Source: CAD feature listing. Evaluate the final solid. Frame: model axes, mm. Face numbers are marked on the shaded views. Give positions to 0.01 mm unless a question says otherwise; leave off trailing zeros. Order: outer loops, then holes, each group sorted by start corner. A loop starts at its lowest first (then second) coordinate and runs counter-clockwise, first axis right, second up.
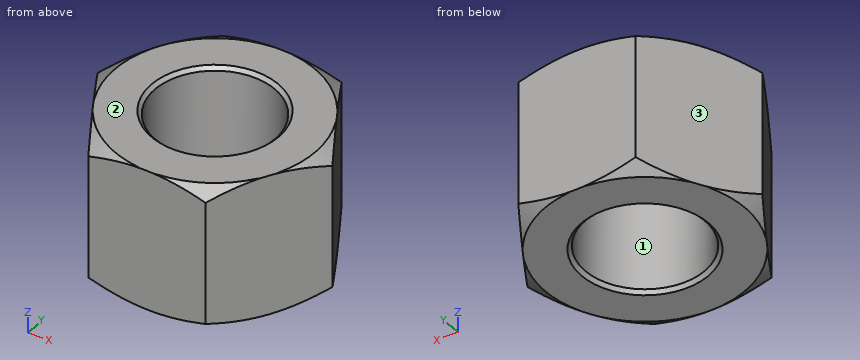
```python
from build123d import *

# Parameters (mm, degrees)
SKETCH1_R          = 5.9175
BOSS_EXTRUDE_DEPTH = 13.9
SKETCH2_OUTSIDE_W  = 105.954
SKETCH2_OUTSIDE_H  = 102.9
SKETCH2_OUTSIDE_R  = 9.872689603
CUT_EXTRUDE1_DEPTH = 21.509509989
CUT_EXTRUDE1_DRAFT = -60
SKETCH3_OUTSIDE_W  = 105.954
SKETCH3_OUTSIDE_H  = 102.9
SKETCH3_OUTSIDE_R  = 9.872689603
CUT_EXTRUDE2_DEPTH = 21.509509989
CUT_EXTRUDE2_DRAFT = -60
CHAMFER1_SIZE      = 0.3475


with BuildPart() as part:
    # Sketch1 → Boss-Extrude (new body)
    with BuildSketch(Plane.XY):
        Polygon((5.7, 9.872689603), (-5.7, 9.872689603), (-11.4, 0), (-5.7, -9.872689603), (5.7, -9.872689603), (11.4, 0), align=None)
        Circle(SKETCH1_R, mode=Mode.SUBTRACT)
    extrude(amount=BOSS_EXTRUDE_DEPTH)


with BuildPart() as cut_extrude1_tool:
    # Sketch2 outside → Cut-Extrude1 (with draft: the straight prism first)
    with BuildSketch(Plane(origin=(0, 0, 0), x_dir=(-1, 0, 0), z_dir=(0, 0, -1))):
        Rectangle(SKETCH2_OUTSIDE_W, SKETCH2_OUTSIDE_H)
        Circle(SKETCH2_OUTSIDE_R, mode=Mode.SUBTRACT)
    extrude(amount=-CUT_EXTRUDE1_DEPTH)
    # Cut-Extrude1: the draft: its side faces are tilted about the plane it starts from
    cut_extrude1_sides = [cut_extrude1_tool.faces().sort_by_distance(p)[0] for p in [
        (0, -51.45, 10.754754995),
        (-52.977, 0, 10.754754995),
        (0, 51.45, 10.754754995),
        (52.977, 0, 10.754754995),
        (9.872689603, 0, 10.754754995),
    ]]
    draft(cut_extrude1_sides, Plane(origin=(0, 0, 0), x_dir=(-1, 0, 0), z_dir=(0, 0, -1)), CUT_EXTRUDE1_DRAFT)


with BuildPart() as part_1:
    add(part.part)

    # Cut-Extrude1: cut by cut_extrude1_tool
    add(cut_extrude1_tool.part, mode=Mode.SUBTRACT)


with BuildPart() as cut_extrude2_tool:
    # Sketch3 outside → Cut-Extrude2 (with draft: the straight prism first)
    with BuildSketch(Plane.XY.offset(13.9)):
        Rectangle(SKETCH3_OUTSIDE_W, SKETCH3_OUTSIDE_H)
        Circle(SKETCH3_OUTSIDE_R, mode=Mode.SUBTRACT)
    extrude(amount=-CUT_EXTRUDE2_DEPTH)
    # Cut-Extrude2: the draft: its side faces are tilted about the plane it starts from
    cut_extrude2_sides = [cut_extrude2_tool.faces().sort_by_distance(p)[0] for p in [
        (0, -51.45, 3.145245005),
        (52.977, 0, 3.145245005),
        (0, 51.45, 3.145245005),
        (-52.977, 0, 3.145245005),
        (-9.872689603, 0, 3.145245005),
    ]]
    draft(cut_extrude2_sides, Plane.XY.offset(13.9), CUT_EXTRUDE2_DRAFT)


with BuildPart() as part_2:
    add(part_1.part)

    # Cut-Extrude2: cut by cut_extrude2_tool
    add(cut_extrude2_tool.part, mode=Mode.SUBTRACT)

    # Chamfer1
    chamfer1_edges = [part_2.edges().sort_by_distance(p)[0] for p in [
        (-5.9175, 0, 0),
        (-5.9175, 0, 13.9),
    ]]
    chamfer(chamfer1_edges, length=CHAMFER1_SIZE)


solid = part_2.part
```
1) Section query A-A, the plane z = 4.25. Return the cut outline in (x, y) (1 decimal).
Report:
outline: (-11.4, 0) - (-5.7, -9.9) - (5.7, -9.9) - (11.4, 0) - (5.7, 9.9) - (-5.7, 9.9) - close; hole circle Ø11.8 at (0, 0)
2) Draft query along Y for the marked faces 1, 2 and 3. Return one class per face: +Y half, -Y half, draft (parallel to the pull), parting line (faces both ways), or undercut.
Report:
face 1: undercut
face 2: draft
face 3: +Y half
3) Pin query (flat end, axial travel): pin 1 (8 mm diameter, centred on y = -7, z = 6, fed in from +X); pin 2 (9.5 mm diameter, centred on x = 0, y = 0, fed in from -Z); pin 3 (6 mm diameter, centred on y = 2.5, z = 6.5, fed in from -X); pin 4 (3 mm diameter, centred on x = -8.5, z = 7, fed in from +Y). Return the tip coordinate at first contact, or that it passes through.
Report:
pin 1: stops at x = 9.67
pin 2: passes through
pin 3: stops at x = -11.4
pin 4: stops at y = 7.62
4) Material intervals for L1, parallel to Y at x = 0, z = 4.5; L2, parallel to Y at x = -1.5, z = 10.75; L3, parallel to X at y = 1, z = 5, sorted ascending.
Report:
L1: y = -9.87 to -5.92, 5.92 to 9.87
L2: y = -9.87 to -5.72, 5.72 to 9.87
L3: x = -10.82 to -5.83, 5.83 to 10.82
